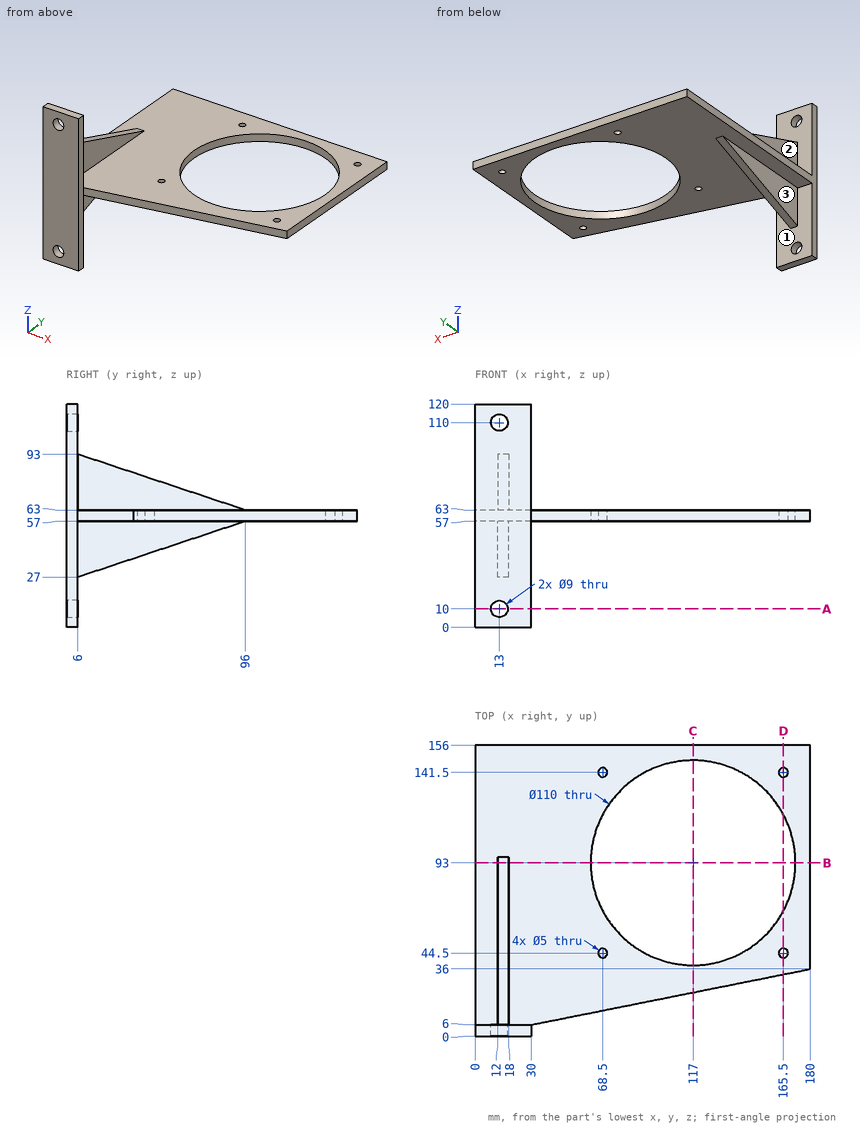
Design review of the part shown in the three views and the two pictorial views. Dimensions are in mm from the part's minimum x, y and z. A direction names the side the tool comes from. Round coordinates to 2 decimals unless told otherwise and drop trailing zeros. Write each loop counter-clockwise with the first axis right and the second up, starting at its lowest first coordinate (ties: lowest second). Pieces come first, ordered by that corner, then holes. Notation, with made-up numbers: (0, 24) - (7, 24) arc R34 cw to (7, 60) - close; hole circle Ø11 at (58, -3.5). An arc over 180 degrees is marked (long way). Write item = value, one per line. Start each with the question number.
1. Consider section C-C on x = 117. State the section outline as (y, z) points.
2. For pin 1 Ø6.5 at (x, y) = (165.5, 44.5) entering from +Z; pin 2 Ø15 at (y, z) = (35.5, 76.5) entering from +X; pin 3 Ø4.5 at (x, y) = (68.5, 44.5) entering from +Z; pin 4 Ø12 at (x, z) = (83.5, 54) entering from -Y, all flat-tipped, find the tip position at first contact; note any pin that passes through.
3. Wall thickness on L1, parallel to Y at x = 68, z = 61; L2, parallel to X at y = 141.5, z = 60.95; L3, parallel to X at y = 24, z = 50.5: over which ranges is each line inside the solid? List them lowest first.
4. Consider section A-A on z = 10. State the section outline as (x, y) points, plus the area to 3 significant figures.
5. Consider section D-D on x = 165.5. State the section outline as (y, z) points.
6. Consider section B-B on y = 93. State the section outline as (x, z) points.
7. For the marked faces 1, 2 and 3, list the 3-axis set-ups (+Z, -Z, +X, -X, +Y, -Y) from which the entire face can be reached by the end or side of a thin tool; tool diameter is ignored.
Evaluation:
q1.outline = (23.4, 57) - (38, 57) - (38, 63) - (23.4, 63) - close; (148, 57) - (156, 57) - (156, 63) - (148, 63) - close
q2.pin_1 = 63
q2.pin_2 = 18
q2.pin_3 = through
q2.pin_4 = 15.66
q3.L1 = 13.6 to 42.05, 46.95 to 68.02, 117.98 to 139.05, 143.95 to 156
q3.L2 = 0 to 66, 71 to 91.06, 142.94 to 163, 168 to 180
q3.L3 = 12 to 18
q4.outline = (0, 0) - (8.5, 0) - (8.5, 6) - (0, 6) - close; (17.5, 0) - (30, 0) - (30, 6) - (17.5, 6) - close
q4.area = 126 mm2
q5.outline = (33.1, 57) - (42, 57) - (42, 63) - (33.1, 63) - close; (47, 57) - (67.06, 57) - (67.06, 63) - (47, 63) - close; (118.94, 57) - (139, 57) - (139, 63) - (118.94, 63) - close; (144, 57) - (156, 57) - (156, 63) - (144, 63) - close
q6.outline = (0, 57) - (12, 57) - (12, 56) - (18, 56) - (18, 57) - (62, 57) - (62, 63) - (18, 63) - (18, 64) - (12, 64) - (12, 63) - (0, 63) - close; (172, 57) - (180, 57) - (180, 63) - (172, 63) - close
q7.face_1 = -Z, +Y
q7.face_2 = +Z, -X, +Y
q7.face_3 = -Z, -X, +Y
